Geometry check sheet. Reference: the model listing, model coordinates, mm. A direction names the side the tool comes from. Coordinates: 2 decimals unless noted, no trailing zeros. Order: outer loops, then holes, each group sorted by start corner. A loop starts at its lowest first (then second) coordinate and runs counter-clockwise, first axis right, second up.
```python
from build123d import *

# Parameters (mm, degrees)
SKETCH1_R           = 45
SKETCH1_R_2         = 14
BOSS_EXTRUDE1_DEPTH = 8
SKETCH2_R           = 41
SKETCH2_R_2         = 37
SKETCH2_R_3         = 23
SKETCH2_R_4         = 19
CUT_EXTRUDE1_DEPTH  = 2
CUT_EXTRUDE2_DEPTH  = 100
CUT_EXTRUDE3_DEPTH  = 4
CUT_EXTRUDE4_DEPTH  = 2


with BuildPart() as part:
    # Sketch1 → Boss-Extrude1 (new body)
    with BuildSketch(Plane.XY):
        Circle(SKETCH1_R)
        Circle(SKETCH1_R_2, mode=Mode.SUBTRACT)
    extrude(amount=BOSS_EXTRUDE1_DEPTH)

    # Sketch2 → Cut-Extrude1 (cut)
    # profile 1 of 4: a face of its own
    with BuildSketch(Plane.XY.offset(8)):
        Circle(SKETCH2_R)
        Circle(SKETCH2_R_2, mode=Mode.SUBTRACT)
    # profile 2 of 4: a face of its own
    with BuildSketch(Plane.XY.offset(8)):
        Circle(SKETCH2_R_3)
        Circle(SKETCH2_R_4, mode=Mode.SUBTRACT)
    # profile 3 of 4: a face of its own
    with BuildSketch(Plane.XY.offset(8)):
        with BuildLine():
            ThreePointArc((31.392589354, 8.411618966), (0, 32.5), (-31.392589354, 8.411618966))
            ThreePointArc((-31.392589354, 8.411618966), (-29.624822401, 5.349756787), (-26.562960223, 7.11752374))
            ThreePointArc((-26.562960223, 7.11752374), (0, 27.5), (26.562960223, 7.11752374))
            ThreePointArc((26.562960223, 7.11752374), (29.624822401, 5.349756787), (31.392589354, 8.411618966))
        make_face()
    # profile 4 of 4: a face of its own
    with BuildSketch(Plane.XY.offset(8)):
        with BuildLine():
            ThreePointArc((-31.392589354, -8.411618966), (-29.624822401, -5.349756787), (-26.562960223, -7.11752374))
            ThreePointArc((-26.562960223, -7.11752374), (0, -27.5), (26.562960223, -7.11752374))
            ThreePointArc((26.562960223, -7.11752374), (29.624822401, -5.349756787), (31.392589354, -8.411618966))
            ThreePointArc((31.392589354, -8.411618966), (0, -32.5), (-31.392589354, -8.411618966))
        make_face()
    extrude(amount=-CUT_EXTRUDE1_DEPTH, mode=Mode.SUBTRACT)

    # Sketch3 → Cut-Extrude2 (cut)
    with BuildSketch(Plane.XY.offset(6)):
        with BuildLine():
            ThreePointArc((31.392589354, 8.411618966), (0, 32.5), (-31.392589354, 8.411618966))
            ThreePointArc((-31.392589354, 8.411618966), (-29.624822401, 5.349756787), (-26.562960223, 7.11752374))
            ThreePointArc((-26.562960223, 7.11752374), (0, 27.5), (26.562960223, 7.11752374))
            ThreePointArc((26.562960223, 7.11752374), (29.624822401, 5.349756787), (31.392589354, 8.411618966))
        make_face()
        with BuildLine():
            ThreePointArc((-26.562960223, -7.11752374), (-29.624822401, -5.349756787), (-31.392589354, -8.411618966))
            ThreePointArc((-31.392589354, -8.411618966), (0, -32.5), (31.392589354, -8.411618966))
            ThreePointArc((31.392589354, -8.411618966), (29.624822401, -5.349756787), (26.562960223, -7.11752374))
            ThreePointArc((26.562960223, -7.11752374), (0, -27.5), (-26.562960223, -7.11752374))
        make_face()
    extrude(amount=-CUT_EXTRUDE2_DEPTH, mode=Mode.SUBTRACT)

    # Sketch4<3> → Cut-Extrude3 (cut)
    with BuildSketch(Plane.XY.offset(8)):
        with BuildLine():
            Line((-45, -2.5), (-40, -2.5))
            ThreePointArc((-40, -2.5), (-37.5, 0), (-40, 2.5))
            Line((-40, 2.5), (-45, 2.5))
            ThreePointArc((-45, 2.5), (-47.5, 0), (-45, -2.5))
        make_face()
        with BuildLine():
            ThreePointArc((40, -2.5), (37.5, 0), (40, 2.5))
            Line((40, 2.5), (45, 2.5))
            ThreePointArc((45, 2.5), (47.5, 0), (45, -2.5))
            Line((45, -2.5), (40, -2.5))
        make_face()
    extrude(amount=-CUT_EXTRUDE3_DEPTH, mode=Mode.SUBTRACT)

    # 草图4<3> → Cut-Extrude4 (cut)
    with BuildSketch(Plane.XY.offset(8)):
        with BuildLine():
            Line((22.912878475, -2), (36.945906404, -2))
            ThreePointArc((36.945906404, -2), (36.986474129, -1.000365698), (37, 0))
            ThreePointArc((37, 0), (36.986474129, 1.000365698), (36.945906404, 2))
            Line((36.945906404, 2), (22.912878475, 2))
            ThreePointArc((22.912878475, 2), (22.978209296, 1.00094832), (23, 0))
            ThreePointArc((23, 0), (22.978209296, -1.00094832), (22.912878475, -2))
        make_face()
        with BuildLine():
            ThreePointArc((-36.945906404, 2), (-37, 0), (-36.945906404, -2))
            Line((-36.945906404, -2), (-22.912878475, -2))
            ThreePointArc((-22.912878475, -2), (-23, 0), (-22.912878475, 2))
            Line((-22.912878475, 2), (-36.945906404, 2))
        make_face()
        with BuildLine():
            Line((22.912878475, -2), (36.945906404, -2))
            ThreePointArc((36.945906404, -2), (36.986474129, -1.000365698), (37, 0))
            ThreePointArc((37, 0), (36.986474129, 1.000365698), (36.945906404, 2))
            Line((36.945906404, 2), (22.912878475, 2))
            ThreePointArc((22.912878475, 2), (22.978209296, 1.00094832), (23, 0))
            ThreePointArc((23, 0), (22.978209296, -1.00094832), (22.912878475, -2))
        make_face()
        with BuildLine():
            ThreePointArc((-36.945906404, 2), (-37, 0), (-36.945906404, -2))
            Line((-36.945906404, -2), (-22.912878475, -2))
            ThreePointArc((-22.912878475, -2), (-23, 0), (-22.912878475, 2))
            Line((-22.912878475, 2), (-36.945906404, 2))
        make_face()
    extrude(amount=-CUT_EXTRUDE4_DEPTH, mode=Mode.SUBTRACT)


solid = part.part
```
Item 1: Sectioned sample at A-A (x = 0). Give the number of separate pieces and of enclosed holes in the cut face, and give its area (3 significant figures).
Item 2: Sectioned sample at B-B (y = 0). Record the cut outline in (x, z).
Item 3: Sectioned sample at C-C (x = 25). Record the cut outline in (y, z), and give its area (3 significant figures).
Item 4: Tool access check on faces 1 (the face through (41, 0, 4)), 2 (the face through (-4, -41, 8)), 3 (the face through (0.596, 32.495, 4.056)), 4 (the face through (0.79, 36.99, 7.01)). Record the directions out of +Z, -Z, +X, -X, +Y, -Y that give a thin tool (end or side, any length) a straight path to the whole face; none if there is none.
Item 5: Depth check by flat-ended pin: P1, Ø2, axis at y = -3, z = 6, coming from the +X side; P2, Ø5.5, axis at x = -42, y = 0.5, coming from the +Z side; P3, Ø1.2, axis at x = 41.5, z = 6, coming from the -Y side; P4, Ø0.6, axis at x = 32, z = 7, coming from the +Y side. Enter the tip coordinate at first touch or a pass-through.
Item 6: Sectioned sample at D-D (y = -16.5). Record the cut outline in (x, z), and give its area (3 significant figures).
Item 7: Thickness scan on line 1 along Y through (x, z) = (-22, 4); line 2 along Y through (x, z) = (25.5, 6.25); line 3 along Y through (x, z) = (10, 3.5). Record the ranges inside material, lowest first.
Item 8: Release check for a two-part mould opening along X. For faces 5 (the face through (-30, 2, 7)), 6 (the face through (-37.5, -0.1, 5)), 7 (the face through (-0.596, -32.495, 4.056)) record: pulls with the +X half, pulls with the -X half, needs draft (parallel to the pull), parting line crosses it, or undercut.
Geometry check:
1. separate pieces: 4
1. enclosed holes: 0
1. area: 384 mm2
2. outline: (-45, 0) - (-14, 0) - (-14, 8) - (-19, 8) - (-19, 6) - (-37.5, 6) - (-37.5, 4) - (-45, 4) - close; (14, 0) - (45, 0) - (45, 4) - (37.5, 4) - (37.5, 6) - (19, 6) - (19, 8) - (14, 8) - close
3. outline: (-37.42, 0) - (-20.77, 0) - (-20.77, 8) - (-27.28, 8) - (-27.28, 6) - (-32.5, 6) - (-32.5, 8) - (-37.42, 8) - close; (-11.46, 0) - (11.46, 0) - (11.46, 8) - (2, 8) - (2, 6) - (-2, 6) - (-2, 8) - (-11.46, 8) - close; (20.77, 0) - (37.42, 0) - (37.42, 8) - (32.5, 8) - (32.5, 6) - (27.28, 6) - (27.28, 8) - (20.77, 8) - close
3. area: 421 mm2
4. face 1: +Z, +X
4. face 2: +Z, +X, -X, +Y, -Y
4. face 3: +Z, -Z
4. face 4: +Z
5. P1: stops at x = 44.93
5. P2: stops at z = 8
5. P3: stops at y = -18.77
5. P4: stops at y = 31.94
6. outline: (-41.87, 0) - (-28, 0) - (-28, 8) - (-33.12, 8) - (-33.12, 6) - (-37.53, 6) - (-37.53, 8) - (-41.87, 8) - close; (-22, 0) - (22, 0) - (22, 8) - (16.02, 8) - (16.02, 6) - (9.42, 6) - (9.42, 8) - (-9.42, 8) - (-9.42, 6) - (-16.02, 6) - (-16.02, 8) - (-22, 8) - close; (28, 0) - (41.87, 0) - (41.87, 8) - (37.53, 8) - (37.53, 6) - (33.12, 6) - (33.12, 8) - (28, 8) - close
6. area: 530 mm2
7. line 1: y = -39.26 to -23.92, -16.5 to 16.5, 23.92 to 39.26
7. line 2: y = -37.08 to -32.11, -26.81 to -20.15, -10.3 to -2, 2 to 10.3, 20.15 to 26.81, 32.11 to 37.08
7. line 3: y = -43.87 to -30.92, -25.62 to -9.8, 9.8 to 25.62, 30.92 to 43.87
8. face 5: needs draft
8. face 6: pulls with the -X half
8. face 7: undercut
